Can you work these out from the drawing? Everything is in mm from the part's minimum corner. A direction names the side the tool comes from. Round coordinates to 2 decimals unless told otherwise and drop trailing zeros. Write each loop counter-clockwise with the first axis right and the second up, starting at its lowest first coordinate (ties: lowest second). Pieces come first, ordered by that corner, then holes. Notation, with made-up numbers: (61.25, 69) -> (92.25, 69) arc R17 cw to (92.25, 99) -> close; hole circle Ø10 at (85.5, 22). An arc over 180 degrees is marked (long way). Answer as CSV lines item,"result". Start each with the question number.
Q1. If I drill on line 1 (X direction, y = 10.5, z = 33); line 2 (Y direction, x = 10, z = 26.5); line 3 (Z direction, x = 7.25, y = 11), over which ranges is the centre line in solid material (lowest first)? Write a range as [from, to].
Q2. For the marked faces 1, 2 and 3, which set-ups out of +Z, -Z, +X, -X, +Y, -Y let a thin tool reach every point of the face, with its end or its side?
Q3. Imagine slicing it at A-A on x = 9.75. Please give me the cut outline in (y, z).
Q4. Imagine slicing it at D-D on x = 5. Please give me the cut outline in (y, z), and give its area (3 significant figures).
Q5. Will these pins go through, and if not, where does the flat tip stop? pin 1 Ø2 at (y, z) = (46, 29) entering from -X; pin 2 Ø8 at (y, z) = (26.5, 53) entering from -X; pin 3 Ø3 at (x, y) = (4.5, 15) entering from -Z.
Q6. Imagine slicing it at C-C on y = 7.5. Please give me the cut outline in (x, z).
Q7. Imagine slicing it at B-B on z = 12. Please give me the cut outline in (x, y).
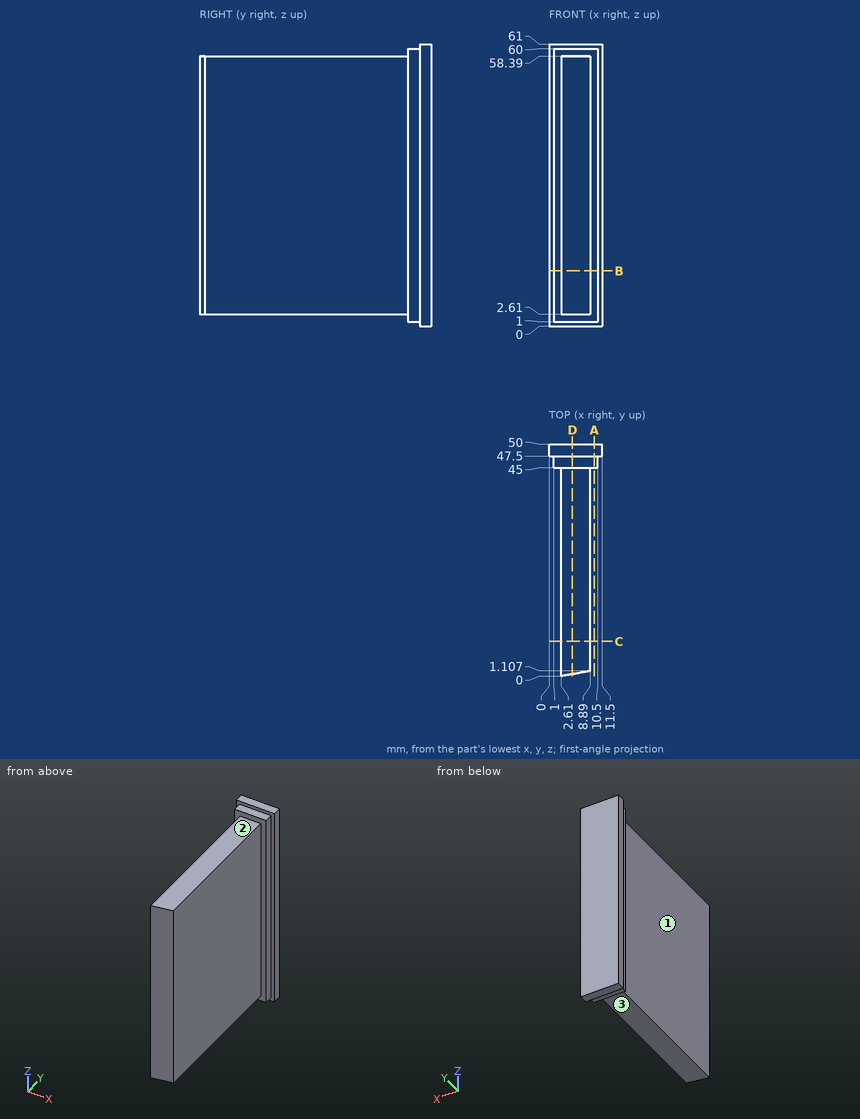
Checks:
1,line 1,"[2.61, 8.89]"
1,line 2,"[45, 50]"
1,line 3,"[2.61, 58.39]"
2,face 1,"+Z, -Z, -X, -Y"
2,face 2,"+Z, +X, -X, -Y"
2,face 3,"-Z, +X, -X, -Y"
3,outline,"(45, 1) -> (47.5, 1) -> (47.5, 0) -> (50, 0) -> (50, 61) -> (47.5, 61) -> (47.5, 60) -> (45, 60) -> close"
4,outline,"(0.42, 2.61) -> (45, 2.61) -> (45, 1) -> (47.5, 1) -> (47.5, 0) -> (50, 0) -> (50, 61) -> (47.5, 61) -> (47.5, 60) -> (45, 60) -> (45, 58.39) -> (0.42, 58.39) -> close"
4,area,"2,790 mm^2"
5,pin 1,"x = 1"
5,pin 2,"x = 2.61"
5,pin 3,"z = 2.61"
6,outline,"(2.61, 2.61) -> (8.89, 2.61) -> (8.89, 58.39) -> (2.61, 58.39) -> close"
7,outline,"(0, 47.5) -> (1, 47.5) -> (1, 45) -> (2.61, 45) -> (2.61, 0) -> (8.89, 1.11) -> (8.89, 45) -> (10.5, 45) -> (10.5, 47.5) -> (11.5, 47.5) -> (11.5, 50) -> (0, 50) -> close"
